Build history of the part. All positions in model axes, mm. Face numbers are marked on the shaded views. A direction names the side the tool comes from. Round coordinates to 2 decimals unless told otherwise and drop trailing zeros. Write each loop counter-clockwise with the first axis right and the second up, starting at its lowest first coordinate (ties: lowest second). Pieces come first, ordered by that corner, then holes. Notation, with made-up numbers: (8, 87) - (63, 87) arc R16 cw to (63, 97) - close; hole circle Ø4 at (19, 1.5). An arc over 180 degrees is marked (long way). Answer as a JSON object with one key per item and string values. Group by question number.
Item 1: Slice it at A-A, the plane y = 30. List the corners of the cut face in (x, z), then the cut area to 3 significant figures.
Item 2: Slice it at D-D, the plane y = 17. List the corners of the cut face in (x, z).
Item 3: Slice it at B-B, the plane x = -7.5. List the corners of the cut face in (y, z).
Item 4: Flat gauge pins, fed straight in: pin 1 (6 mm diameter, centred on x = 10, y = -31, fed in from +Z); pin 2 (2 mm diameter, centred on y = -8.5, z = 4, fed in from +X). Where does each tip first touch, or does it go through?
Item 5: Which spindle directions (+Z, -Z, +X, -X, +Y, -Y) get a long thin tool onto all of the face, cutting with end or side? Do the marked faces 1 and 2. Say none if no direction does.
Item 6: Slice it at C-C, the plane z = 1. List the corners of the cut face in (x, y), then the cut area to 3 significant figures.
Item 7: Probe line 1 (Y direction, x = -7.5, z = -1.25); line 2 (Y direction, x = -41.5, z = 3); line 3 (Z direction, x = -23, y = 3). List the from-to ranges inside material, lowest first. Write a range as from..to.
from build123d import *

# Parameters (mm, degrees)
SKETCH_1_W             = 105
SKETCH_1_H             = 80
EXTRUDE_1_DEPTH        = 5
SKETCH_2_W             = 80
SKETCH_2_H             = 80
CUT_EXTRUDE_1_DEPTH    = 2.5
HOLE_WIZARD_9_0_9_1_D  = 9
HOLE_WIZARD_7_0_7_1_D  = 7
CHAMFER_1_SIZE         = 2
CUT_EXTRUDE_3_DEPTH    = 10
PATTERN_LINEAR_1_COUNT = 2
PATTERN_LINEAR_1_PITCH = 60


with BuildPart() as part:
    # 草图1 → 凸台-拉伸1 (new, symmetric)
    with BuildSketch(Plane.XY):
        Rectangle(SKETCH_1_W, SKETCH_1_H)
    extrude(amount=EXTRUDE_1_DEPTH, both=True)

    # 草图2 → 切除-拉伸1 (cut)
    with BuildSketch(Plane.XY.offset(5)):
        with Locations((12.5, 0)):
            Rectangle(SKETCH_2_W, SKETCH_2_H)
    extrude(amount=-CUT_EXTRUDE_1_DEPTH, mode=Mode.SUBTRACT)

    # Ø9.0 (9) 直径孔1 (through all)
    with Locations(Plane.XY.offset(5)):
        with Locations((-7.5, 30), (32.5, 30), (32.5, -30), (-7.5, -30)):
            Hole(HOLE_WIZARD_9_0_9_1_D / 2)

    # Ø7.0 (7) 直径孔1 (through all)
    with Locations(Plane.XY.offset(5)):
        with Locations((-44, 30), (-86, 30), (-44, -30), (-86, -30)):
            Hole(HOLE_WIZARD_7_0_7_1_D / 2)

    # 倒角1
    chamfer_1_edges = [part.edges().sort_by_distance(p)[0] for p in [
        (52.5, -40, -1.25),
        (52.5, 40, -1.25),
        (-52.5, -40, 0),
        (-52.5, 40, 0),
    ]]
    chamfer(chamfer_1_edges, length=CHAMFER_1_SIZE)

    # 草图8 → 切除-拉伸3 (cut)
    with BuildSketch(Plane.XY.offset(5)):
        with BuildLine():
            Line((-40, 26.5), (-48, 26.5))
            ThreePointArc((-48, 26.5), (-51.5, 30), (-48, 33.5))
            Line((-48, 33.5), (-40, 33.5))
            ThreePointArc((-40, 33.5), (-36.5, 30), (-40, 26.5))
        make_face()
    cut_extrude_3 = extrude(amount=-CUT_EXTRUDE_3_DEPTH, mode=Mode.SUBTRACT)

    # 阵列(线性)1: 切除-拉伸3 ×2
    with Locations(*[(0, -i * PATTERN_LINEAR_1_PITCH, 0) for i in range(1, PATTERN_LINEAR_1_COUNT)]):
        add(cut_extrude_3, mode=Mode.SUBTRACT)


solid = part.part
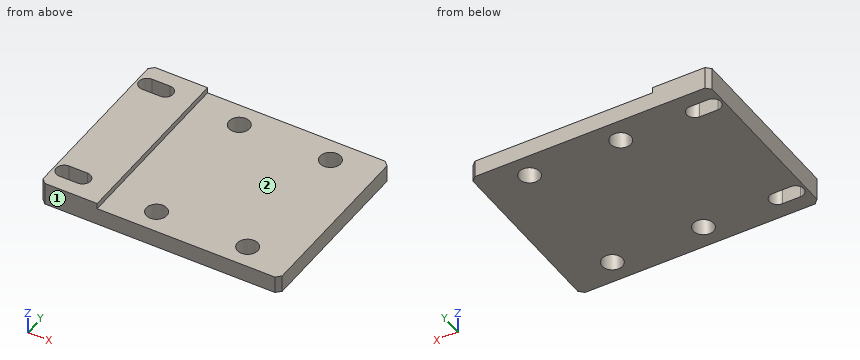
Geometry says:
{
 "1": {"outline": "(-52.5, -5) - (-51.5, -5) - (-51.5, 5) - (-52.5, 5) - close; (-36.5, -5) - (-12, -5) - (-12, 2.5) - (-27.5, 2.5) - (-27.5, 5) - (-36.5, 5) - close; (-3, -5) - (28, -5) - (28, 2.5) - (-3, 2.5) - close; (37, -5) - (52.5, -5) - (52.5, 2.5) - (37, 2.5) - close", "area": "565 mm^2"},
 "2": {"outline": "(-52.5, -5) - (52.5, -5) - (52.5, 2.5) - (-27.5, 2.5) - (-27.5, 5) - (-52.5, 5) - close"},
 "3": {"outline": "(-40, -5) - (-34.5, -5) - (-34.5, 2.5) - (-40, 2.5) - close; (-25.5, -5) - (25.5, -5) - (25.5, 2.5) - (-25.5, 2.5) - close; (34.5, -5) - (40, -5) - (40, 2.5) - (34.5, 2.5) - close"},
 "4": {"pin 1": "stops at z = 2.5", "pin 2": "stops at x = -27.5"},
 "5": {"face 1": "+Z, -Z, +X, -X, -Y", "face 2": "+Z, +X, +Y, -Y"},
 "6": {"outline": "(-52.5, -38) - (-50.5, -40) - (50.5, -40) - (52.5, -38) - (52.5, 38) - (50.5, 40) - (-50.5, 40) - (-52.5, 38) - close; hole (-48, -33.5) - (-40, -33.5) arc R3.5 ccw to (-40, -26.5) - (-48, -26.5) arc R3.5 ccw to start; hole (-48, 26.5) - (-40, 26.5) arc R3.5 ccw to (-40, 33.5) - (-48, 33.5) arc R3.5 ccw to start; hole circle Ø9 at (-7.5, -30); hole circle Ø9 at (-7.5, 30); hole circle Ø9 at (32.5, -30); hole circle Ø9 at (32.5, 30)", "area": "7,950 mm^2"},
 "7": {"line 1": "y = -40..-34.5, -25.5..25.5, 34.5..40", "line 2": "y = -40..-33.5, -26.5..26.5, 33.5..40", "line 3": "z = -5..2.5"}
}
